Work out the finished part from the listing and answer in its coordinate system (mm). Face numbers are marked on the shaded views. A direction names the side the tool comes from. Round coordinates to 2 decimals unless told otherwise and drop trailing zeros. Order: outer loops, then holes, each group sorted by start corner. A loop starts at its lowest first (then second) coordinate and runs counter-clockwise, first axis right, second up. Notation, with made-up numbers: (44, -36.5) - (94, -36.5) arc R13 ccw to (94, -20.5) - close; hole circle Ø10 at (-16, -36.75). An arc over 180 degrees is marked (long way). Answer in a Markdown table with one row per item.
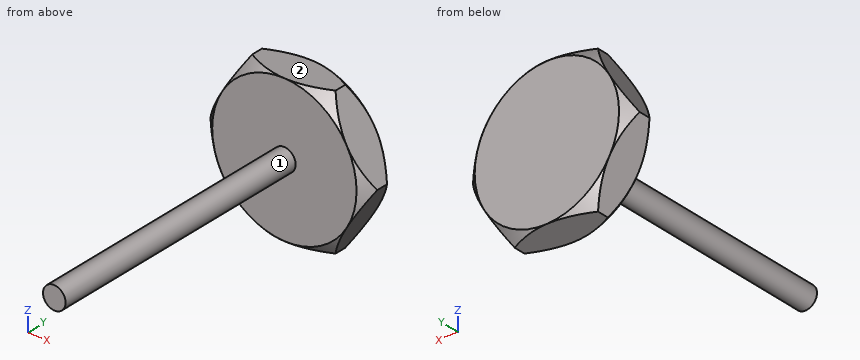
from build123d import *

# Parameters (mm, degrees)
HEX_HEAD_DEPTH                   = 3.75
HEAD_CHAMFER_A_PROFILE_OUTSIDE_W = 32.922
HEAD_CHAMFER_A_PROFILE_OUTSIDE_H = 30.446
HEAD_CHAMFER_A_PROFILE_OUTSIDE_R = 8
HEAD_CHAMFER_A_45DEG_DEPTH       = 3.75
HEAD_CHAMFER_A_45DEG_DRAFT       = -45
HEAD_CHAMFER_B_PROFILE_OUTSIDE_W = 32.922
HEAD_CHAMFER_B_PROFILE_OUTSIDE_H = 30.446
HEAD_CHAMFER_B_PROFILE_OUTSIDE_R = 8
HEAD_CHAMFER_B_45DEG_DEPTH       = 3.75
HEAD_CHAMFER_B_45DEG_DRAFT       = -45
SHANK_PROFILE_2_5_R              = 1.25
SHANK_2_5X30_DEPTH               = 30


with BuildPart() as part:
    # Hex Head Profile → Hex Head (new body)
    with BuildSketch(Plane(origin=(0, 0, 0), x_dir=(1, 0, 0), z_dir=(0, 1, 0))):
        Polygon((4.618802154, -8), (9.237604307, 0), (4.618802154, 8), (-4.618802154, 8), (-9.237604307, 0), (-4.618802154, -8), align=None)
    extrude(amount=HEX_HEAD_DEPTH)


with BuildPart() as head_chamfer_a_45deg_tool:
    # Head Chamfer A Profile outside → Head Chamfer A 45deg (with draft: the straight prism first)
    with BuildSketch(Plane(origin=(0, 3.75, 0), x_dir=(1, 0, 0), z_dir=(0, 1, 0))):
        Rectangle(HEAD_CHAMFER_A_PROFILE_OUTSIDE_W, HEAD_CHAMFER_A_PROFILE_OUTSIDE_H)
        Circle(HEAD_CHAMFER_A_PROFILE_OUTSIDE_R, mode=Mode.SUBTRACT)
    extrude(amount=-HEAD_CHAMFER_A_45DEG_DEPTH)
    # Head Chamfer A 45deg: the draft: its side faces are tilted about the plane it starts from
    head_chamfer_a_45deg_sides = [head_chamfer_a_45deg_tool.faces().sort_by_distance(p)[0] for p in [
        (0, 1.875, 15.223),
        (16.461, 1.875, 0),
        (0, 1.875, -15.223),
        (-16.461, 1.875, 0),
        (-8, 1.875, 0),
    ]]
    draft(head_chamfer_a_45deg_sides, Plane(origin=(0, 3.75, 0), x_dir=(1, 0, 0), z_dir=(0, 1, 0)), HEAD_CHAMFER_A_45DEG_DRAFT)


with BuildPart() as part_1:
    add(part.part)

    # Head Chamfer A 45deg: cut by head_chamfer_a_45deg_tool
    add(head_chamfer_a_45deg_tool.part, mode=Mode.SUBTRACT)


with BuildPart() as head_chamfer_b_45deg_tool:
    # Head Chamfer B Profile outside → Head Chamfer B 45deg (with draft: the straight prism first)
    with BuildSketch(Plane.XZ):
        Rectangle(HEAD_CHAMFER_B_PROFILE_OUTSIDE_W, HEAD_CHAMFER_B_PROFILE_OUTSIDE_H)
        Circle(HEAD_CHAMFER_B_PROFILE_OUTSIDE_R, mode=Mode.SUBTRACT)
    extrude(amount=-HEAD_CHAMFER_B_45DEG_DEPTH)
    # Head Chamfer B 45deg: the draft: its side faces are tilted about the plane it starts from
    head_chamfer_b_45deg_sides = [head_chamfer_b_45deg_tool.faces().sort_by_distance(p)[0] for p in [
        (0, 1.875, -15.223),
        (16.461, 1.875, 0),
        (0, 1.875, 15.223),
        (-16.461, 1.875, 0),
        (-8, 1.875, 0),
    ]]
    draft(head_chamfer_b_45deg_sides, Plane.XZ, HEAD_CHAMFER_B_45DEG_DRAFT)


with BuildPart() as part_2:
    add(part_1.part)

    # Head Chamfer B 45deg: cut by head_chamfer_b_45deg_tool
    add(head_chamfer_b_45deg_tool.part, mode=Mode.SUBTRACT)

    # Shank Profile Ø2.5 → Shank Ø2.5x30 (add)
    with BuildSketch(Plane.XZ):
        with Locations(Location((0, 0, 0), (0, 0, 90))):
            Circle(SHANK_PROFILE_2_5_R)
    extrude(amount=SHANK_2_5X30_DEPTH)


solid = part_2.part
1) Which of the six approach directions +Z, -Z, +X, -X, +Y, -Y give full straight-line access (tool end or side, diameter ignored) to the marked faces 1 and 2?
Filled in:
| item | result |
|---|---|
| face 1 | -Y |
| face 2 | +Z, +X, -X, +Y, -Y |
2) Each of these flat-tipped pins is pushed along its axis until it touches: pin 1 (8 mm diameter, centred on y = -3, z = -2.5, fed in from -X); pin 2 (3 mm diameter, centred on y = -26, z = -3, fed in from -X); pin 3 (10 mm diameter, centred on x = -0.5, y = -25, fed in from -Z); pin 4 (4 mm diameter, centred on y = -3.5, z = -3, fed in from -X). Where does it stop, or does it pass through?
Filled in:
| item | result |
|---|---|
| pin 1 | stops at x = -8.65 |
| pin 2 | passes through |
| pin 3 | stops at z = -1.25 |
| pin 4 | stops at x = -0.75 |
3) Find section A-A, the plane y = -8. Give the vertices of the cut face in (x, z), then the cut area to 3 significant figures.
Filled in:
| item | result |
|---|---|
| outline | circle Ø2.5 at (0, 0) |
| area | 4.91 mm^2 |
4) Find the intervals of material crossed by probe 1 along Y at (x, z) = (-1.25, -2.5); probe 2 along X at (y, z) = (-5, 0); probe 3 along Y at (x, z) = (8, -2), in increasing order. Write a range as from..to.
Filled in:
| item | result |
|---|---|
| probe 1 | y = 0..3.75 |
| probe 2 | x = -1.25..1.25 |
| probe 3 | y = 0.25..3.5 |
